Design review of the part built by this model. Coordinates are the model's own, in mm. Coordinates: 2 decimals unless noted, no trailing zeros. Write each loop counter-clockwise with the first axis right and the second up, starting at its lowest first coordinate (ties: lowest second). Pieces come first, ordered by that corner, then holes. Notation, with made-up numbers: (-39, 40.25) -> (10, 40.25) arc R23 cw to (10, 64.25) -> close; hole circle Ø1 at (8, -5). An arc over 180 degrees is marked (long way). Answer in a Markdown table with one row per item. Add a question column.
Item 1: To check wall thickness, follow line 1 (Y direction, x = 5.25, z = 42). State the ranges of the line that lie inside material, in increasing order.
Item 2: Take a section at B-B, the plane y = 16. Write out the cut boundary in (x, z).
Item 3: Clearance check with flat-ended pins moving along their axes: P1, Ø4, axis at y = 8, z = -66, coming from the +X side; P2, Ø6, axis at x = 7, z = 71, coming from the +Y side. State where each tip first meets the part, or that it passes through.
Item 4: Take a section at A-A, the plane z = 44. Write out the cut boundary in (x, y).
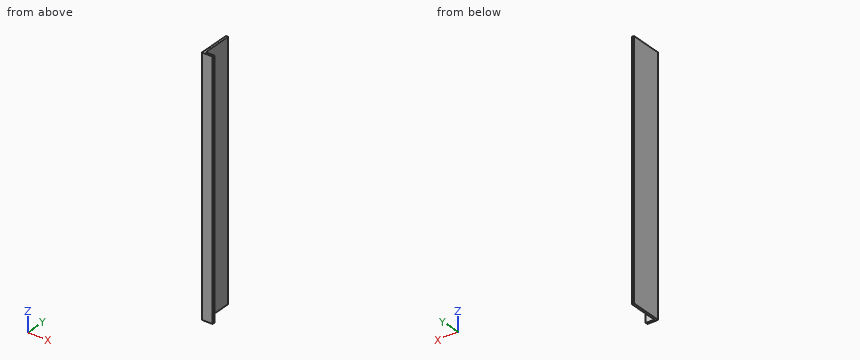
from build123d import *

# Parameters (mm, degrees)
EXTRUDE_1_DEPTH = 116


with BuildPart() as part:
    # 草图1 → 拉伸-薄壁1 (new, symmetric)
    with BuildSketch(Plane.XY):
        Polygon((10, 0), (0, 0), (0, 30), (2, 30), (2, 2), (10, 2), align=None)
    extrude(amount=EXTRUDE_1_DEPTH, both=True)


solid = part.part
Answers:
| question | item | result |
|---|---|---|
| 1 | line 1 | y = 0 to 2 |
| 2 | outline | (0, -116) -> (2, -116) -> (2, 116) -> (0, 116) -> close |
| 3 | P1 | stops at x = 2 |
| 3 | P2 | stops at y = 2 |
| 4 | outline | (0, 0) -> (10, 0) -> (10, 2) -> (2, 2) -> (2, 30) -> (0, 30) -> close |
